from build123d import *

# Parameters (mm, degrees)
EXTRUDE_1_DEPTH     = 50
CHAMFER_1_SIZE      = 3
CUT_EXTRUDE_1_REACH = 136.284
SKETCH_4_R          = 35.5


with BuildPart() as part:
    # 草图2 → 凸台-拉伸1 (new, symmetric)
    with BuildSketch(Plane(origin=(409.637600706, 0.5, -34.379468655), x_dir=(1, 0, 0), z_dir=(0, 0, 1))):
        Polygon((-409.637600706, 96), (-409.637600706, -0.5), (-457.637600706, -0.5), (-457.637600706, 7.5), (-417.637600706, 7.5), (-417.637600706, 96), align=None)
    extrude(amount=EXTRUDE_1_DEPTH, both=True)

    # 倒角1
    chamfer_1_edges = [part.edges().sort_by_distance(p)[0] for p in [
        (-48, 4, 15.620531345),
        (-4, 96.5, 15.620531345),
        (-48, 4, -84.379468655),
        (-4, 96.5, -84.379468655),
    ]]
    chamfer(chamfer_1_edges, length=CHAMFER_1_SIZE)

    # 草图4 → 切除-拉伸1 (cut, up to next)
    with BuildSketch(Plane.ZY.offset(8), mode=Mode.PRIVATE) as cut_extrude_1_sk1:
        with Locations((-34.379468655, 53.5)):
            Circle(SKETCH_4_R)
    cut_extrude_1_tool1 = extrude(cut_extrude_1_sk1.sketch, amount=-CUT_EXTRUDE_1_REACH, mode=Mode.PRIVATE) & part.part
    add(cut_extrude_1_tool1.solids().sort_by_distance((-8, 53.5, -34.379469))[0], mode=Mode.SUBTRACT)


solid = part.part
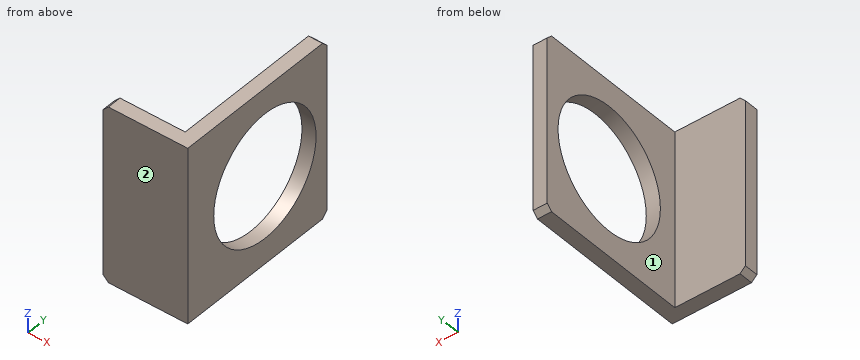
Geometry check sheet. Reference: the model listing, model coordinates, mm. Face numbers are marked on the shaded views. A direction names the side the tool comes from. Give positions to 0.01 mm unless a question says otherwise; leave off trailing zeros. Write each loop counter-clockwise with the first axis right and the second up, starting at its lowest first coordinate (ties: lowest second). Pieces come first, ordered by that corner, then holes. Notation, with made-up numbers: (-31, -17) - (-13, -17) arc R31 cw to (-13, 12) - close; hole circle Ø7 at (77.5, 26). An arc over 180 degrees is marked (long way). Put each result on its own line as item: value.
1. Sectioned sample at D-D, the plane z = -78. Enter the section's corners in (x, y), plus the area to 3 significant figures.
Ans:
outline: (-48, 0) - (0, 0) - (0, 96.5) - (-8, 96.5) - (-8, 8) - (-48, 8) - close
area: 1,090 mm²
2. Sectioned sample at A-A, the plane y = 53.5. Enter the section's corners in (x, z).
Ans:
outline: (-8, -84.38) - (0, -84.38) - (0, -69.88) - (-8, -69.88) - close; (-8, 1.12) - (0, 1.12) - (0, 15.62) - (-8, 15.62) - close
3. Thickness scan on line 1 (X direction, y = 14, z = -63.5); line 2 (Y direction, x = -42, z = -74); line 3 (Y direction, x = -1.5, z = -13). Record the ranges inside material, lowest first.
Ans:
line 1: x = -8 to 0
line 2: y = 0 to 8
line 3: y = 0 to 25.16, 81.84 to 96.5
4. Sectioned sample at B-B, the plane x = -3. Enter the section's corners in (y, z).
Ans:
outline: (0, -84.38) - (93.5, -84.38) - (96.5, -81.38) - (96.5, 12.62) - (93.5, 15.62) - (0, 15.62) - close; hole circle Ø71 at (53.5, -34.38)
5. Go/stop test with flat-tipped pins: pin 1 (5 mm diameter, centred on x = -11.5, y = 77, fed in from +Z); pin 2 (12 mm diameter, centred on x = -26.5, z = -56, fed in from +Y); pin 3 (8 mm diameter, centred on y = 85.5, z = -71.5, fed in from -X). Record where each tip stops, or that it passes through.
Ans:
pin 1: passes through
pin 2: stops at y = 8
pin 3: stops at x = -8
6. Sectioned sample at C-C, the plane z = -28. Enter the section's corners in (x, y).
Ans:
outline: (-48, 0) - (0, 0) - (0, 18.58) - (-8, 18.58) - (-8, 8) - (-48, 8) - close; (-8, 88.42) - (0, 88.42) - (0, 96.5) - (-8, 96.5) - close
7. Set-up check for the marked faces 1 and 2: record each of +Z, -Z, +X, -X, +Y, -Y from which the full face is reachable in a straight line by a thin tool's end or side.
Ans:
face 1: +Z, -Z, -X, +Y
face 2: +Z, -Z, +X, -X, -Y
